The figure shows three views and two pictorial views of one solid part (mm, origin at its lowest corner). Answer the questions. Give positions to 0.01 mm unless a question says otherwise; leave off trailing zeros. Order: outer loops, then holes, each group sorted by start corner. A loop starts at its lowest first (then second) coordinate and runs counter-clockwise, first axis right, second up. Notation, with made-up numbers: M -37.5,31 L -11.5,31 A10 ccw -11.5,45 Z; hole C 26.5,1 d2. An arc over 180 degrees is marked long. One line per item, written item: value. Start each with the question number.
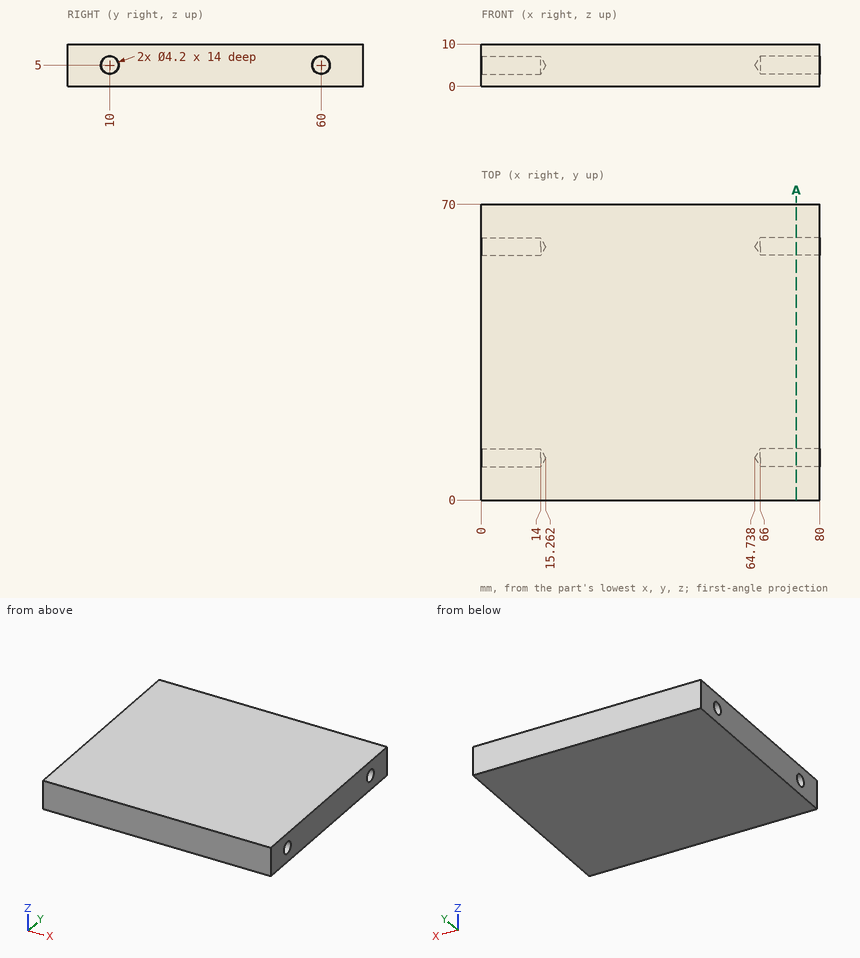
Q1. Consider probe 1 along Y at (x, z) = (76, 5); probe 2 along Z at (x, y) = (71, 60); probe 3 along Y at (x, z) = (10, 4). Determine where each line is inside the solid, lowest interval first.
Q2. Find section A-A, the plane x = 74.5. Give the vertices of the cut face in (y, z), then the cut area to 3 significant figures.
Q3. Each of these flat-tipped pins is pushed along its axis until it touches: pin 1 (4 mm diameter, centred on y = 60, z = 5, fed in from +X); pin 2 (2.5 mm diameter, centred on y = 60, z = 5, fed in from +X). Where does it stop, or does it pass through?
Evaluation:
1. probe 1: 0 to 7.9, 12.1 to 57.9, 62.1 to 70
1. probe 2: 0 to 2.9, 7.1 to 10
1. probe 3: 0 to 8.15, 11.85 to 58.15, 61.85 to 70
2. outline: M 0,0 L 70,0 L 70,10 L 0,10 Z; hole C 10,5 d4.2; hole C 60,5 d4.2
2. area: 672 mm2
3. pin 1: x = 65.94
3. pin 2: x = 65.49
